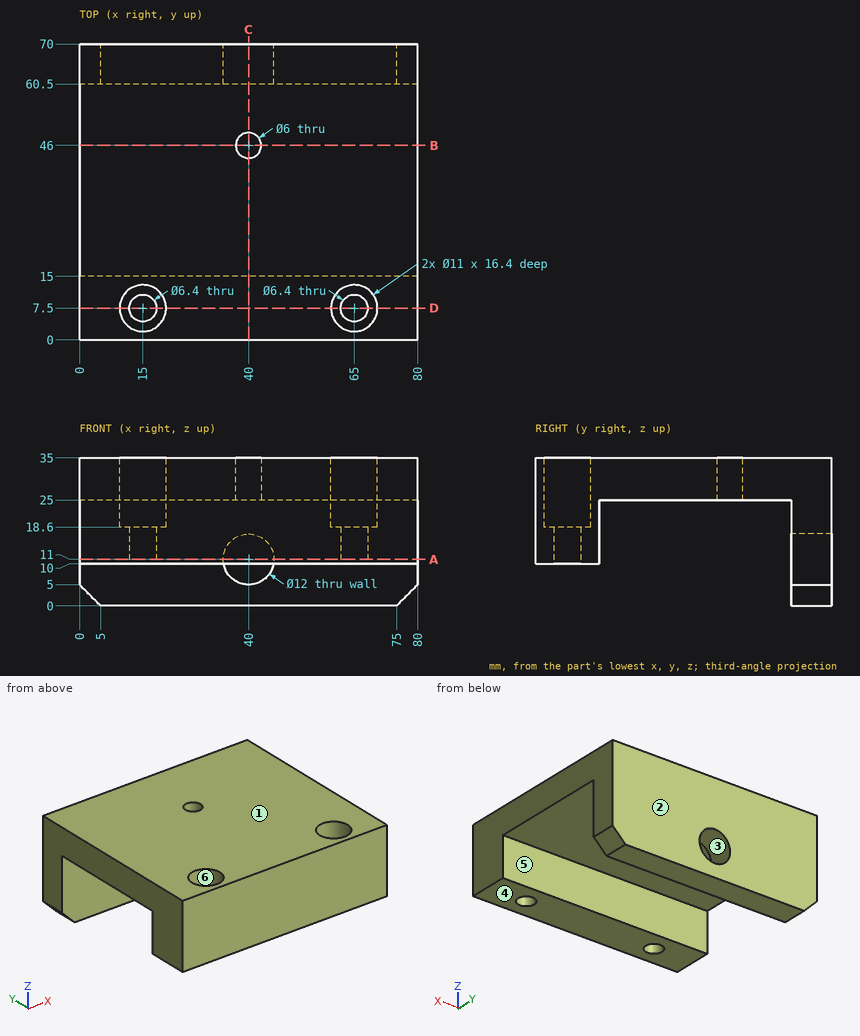
Job drawing, mm, ordinate dimensions from the low corner. One solid piece. A direction names the side the tool comes from. Give positions to 0.01 mm unless a question says otherwise; leave off trailing zeros. Loops run counter-clockwise (first coordinate to the right, second up) from the corner with the lowest first, then second, coordinate; pieces in that order, holes last. Notation, with made-up numbers: M 44,14.5 L 52,14.5 A15 cw 52,19.5 Z; hole C -31,-16 d5. An arc over 180 degrees is marked long. Return JSON: item names as keys, results as strings.
1) Saw through at B-B, the plane y = 46. List the corners of the cut face in (x, z), then the cut area to 3 significant figures.
Calculated:
{"outline": "M 0,25 L 37,25 L 37,35 L 0,35 Z; M 43,25 L 80,25 L 80,35 L 43,35 Z", "area": "740 mm2"}
2) Flat gauge pins, fed straight in: pin 1 Ø6 at (x, y) = (37.5, 53) entering from -Z; pin 2 Ø5.5 at (x, y) = (13, 6.5) entering from +Z; pin 3 Ø11 at (x, z) = (40, 11) entering from +Y. Where does each tip first touch, or does it go through?
Calculated:
{"pin 1": "stops at z = 25", "pin 2": "stops at z = 18.6", "pin 3": "stops at y = 15"}
3) Saw through at D-D, the plane y = 7.5. List the corners of the cut face in (x, z).
Calculated:
{"outline": "M 0,10 L 11.8,10 L 11.8,18.6 L 9.5,18.6 L 9.5,35 L 0,35 Z; M 18.2,10 L 61.8,10 L 61.8,18.6 L 59.5,18.6 L 59.5,35 L 20.5,35 L 20.5,18.6 L 18.2,18.6 Z; M 68.2,10 L 80,10 L 80,35 L 70.5,35 L 70.5,18.6 L 68.2,18.6 Z"}
4) Saw through at C-C, the plane x = 40. List the corners of the cut face in (y, z).
Calculated:
{"outline": "M 0,10 L 15,10 L 15,25 L 43,25 L 43,35 L 0,35 Z; M 49,25 L 60.5,25 L 60.5,17 L 70,17 L 70,35 L 49,35 Z; M 60.5,0 L 70,0 L 70,5 L 60.5,5 Z"}
5) Saw through at A-A, the plane z = 11. List the corners of the cut face in (x, y).
Calculated:
{"outline": "M 0,0 L 80,0 L 80,15 L 0,15 Z; M 0,60.5 L 34,60.5 L 34,70 L 0,70 Z; M 46,60.5 L 80,60.5 L 80,70 L 46,70 Z; hole C 15,7.5 d6.4; hole C 65,7.5 d6.4"}
6) 3-axis set-ups, long thin cutter, end or side, ignore diameter. For the marked faces 4, 5 and 6: which of +Z, -Z, +X, -X, +Y, -Y reach the whole face in a straight line?
Calculated:
{"face 4": "-Z, +X, -X, -Y", "face 5": "-Z, +X, -X", "face 6": "+Z"}
7) Drill centre lines: line 1 (Y direction, x = 15, z = 13); line 2 (Y direction, x = 15, z = 24.75); line 3 (X direction, y = 64.5, z = 10.5). Where is each one in solid material? Low to high.
Calculated:
{"line 1": "y = 0 to 4.3, 10.7 to 15, 60.5 to 70", "line 2": "y = 0 to 2, 13 to 15, 60.5 to 70", "line 3": "x = 0 to 34.02, 45.98 to 80"}
8) Pull direction Z, two halves, no side cores. Call the marked faces 1, 2 and 3: released by +Z, released by -Z, zero draft, split by the parting line, or undercut.
Calculated:
{"face 1": "released by +Z", "face 2": "zero draft", "face 3": "undercut"}
